Part print with two shaded views. Sizes in mm from the minimum x, y, z corner. A direction names the side the tool comes from. Coordinates: 2 decimals unless noted, no trailing zeros. Loops run counter-clockwise (first coordinate to the right, second up) from the corner with the lowest first, then second, coordinate; pieces in that order, holes last.
(1) Slice it at C-C (z = 115). Give the cut face in (x, y), and give its area (3 significant figures).
(2) Slice it at A-A (y = 16). Give the cut face in (x, z), and give its area (3 significant figures).
(3) Slice it at B-B (z = 34). Give the cut face in (x, y), and give its area (3 significant figures).
(4) Wall check: L1, parallel to Y at x = 114.5, z = 50; L2, parallel to Z at x = 26, y = 6; L3, parallel to X at y = 132, z = 108. Give the ranges that are in metal, low to high.
(5) Two-plate mould, pull along X, no slides. Class the marked faces 3, 4 and 5: pulls with the +X half, pulls with the -X half, needs draft (parallel to the pull), parting line crosses it, or undercut.
(6) Slice it at D-D (x = 105). Give the cut face in (y, z).
(7) Tool access for the marked faces 1 and 2: list every direction of +Z, -Z, +X, -X, +Y, -Y with a clear straight run to the whole face (end or side of a thin tool).
(8) Flat gauge pin, fed straight in: P1, Ø10, axis at x = 94, z = 27.5, coming from the +Y side. Where does the tip first touch, or does it go through?
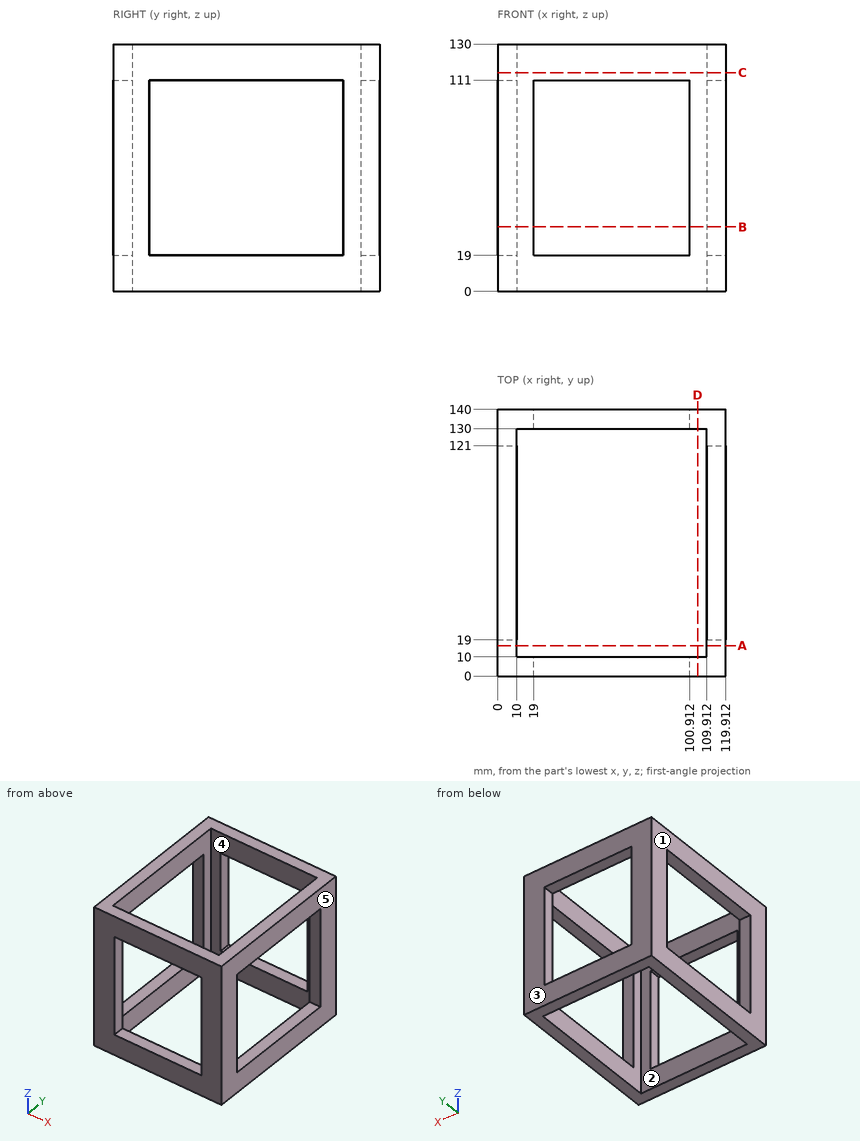
Response values:
1. outline: (0, 0) - (119.91, 0) - (119.91, 140) - (0, 140) - close; hole (10, 10) - (109.91, 10) - (109.91, 130) - (10, 130) - close
1. area: 4,800 mm2
2. outline: (0, 0) - (10, 0) - (10, 130) - (0, 130) - close; (109.91, 0) - (119.91, 0) - (119.91, 130) - (109.91, 130) - close
2. area: 2,600 mm2
3. outline: (0, 0) - (19, 0) - (19, 10) - (10, 10) - (10, 19) - (0, 19) - close; (0, 121) - (10, 121) - (10, 130) - (19, 130) - (19, 140) - (0, 140) - close; (100.91, 0) - (119.91, 0) - (119.91, 19) - (109.91, 19) - (109.91, 10) - (100.91, 10) - close; (100.91, 130) - (109.91, 130) - (109.91, 121) - (119.91, 121) - (119.91, 140) - (100.91, 140) - close
3. area: 1,120 mm2
4. L1: y = 0 to 19, 121 to 140
4. L2: z = 0 to 19, 111 to 130
4. L3: x = 0 to 19, 100.91 to 119.91
5. face 3: needs draft
5. face 4: undercut
5. face 5: pulls with the +X half
6. outline: (0, 0) - (10, 0) - (10, 130) - (0, 130) - close; (130, 0) - (140, 0) - (140, 130) - (130, 130) - close
7. face 1: +Z, -Z, -X, +Y, -Y
7. face 2: +Z, -Z
8. P1: passes through
